Study the drawing (mm; zero at the part's minimum x, y, z) and answer. Coordinates: 2 decimals unless noted, no trailing zeros. Loops run counter-clockwise (first coordinate to the right, second up) from the corner with the lowest first, then second, coordinate; pieces in that order, holes last. Notation, with made-up numbers: (26.25, -23) -> (81.25, -23) arc R36 ccw to (81.25, 16) -> close; hole circle Ø1 at (29, -6). An arc over 180 degrees is marked (long way). Answer as a JSON object with one key per item and string values. Group by question number.
Q1. Straight lines are drawn through the part: line 1 along X through (y, z) = (11.5, 4.85); line 2 along X through (y, z) = (7.75, 3); line 3 along Y through (x, z) = (17.5, 4) (1 decimal). For each, find the intervals that lie inside material, in ascending order. Write a range as [from, to].
Q2. Each of these flat-tipped pins is pushed along its axis until it touches: P1, Ø1, axis at y = 14, z = 6, coming from the -X side (1 decimal); P2, Ø3, axis at x = 17, y = 5.5, coming from the -Z side; P3, Ø0.7, axis at y = 22, z = 4, coming from the +X side (1 decimal); P4, Ø4, axis at y = 8.5, z = 2.5, coming from the +X side. Where does it stop, or does it pass through?
Q3. The part is cut by section C-C on z = 2.5. Write down the section's boundary in (x, y).
Q4. The part is cut by section A-A on y = 11.5. Write down the section's boundary in (x, z), and give its area (3 significant figures).
Q5. The part is cut by section B-B on x = 11.5. Write down the section's boundary in (y, z).
Q6. Determine the mould class of the marked faces 1 and 2 for opening direction Y: released by +Y, released by -Y, zero draft, split by the parting line, or undercut.
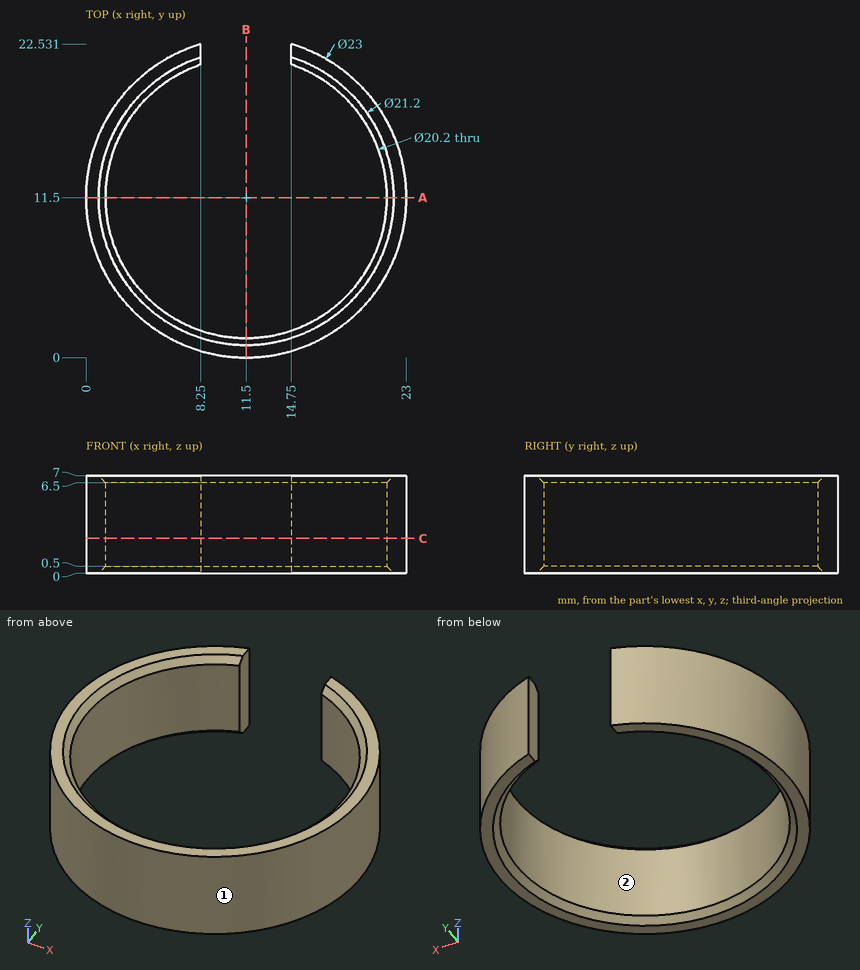
Final values:
{
 "1": {"line 1": "x = [0, 1.4], [21.6, 23]", "line 2": "x = [0.63, 2.12], [20.88, 22.37]", "line 3": "y = [1.7, 3.4], [19.6, 21.3]"},
 "2": {"P1": "stops at x = 0.2", "P2": "passes through", "P3": "stops at x = 16.9", "P4": "stops at x = 22.96"},
 "3": {"outline": "(8.25, 21.06) -> (8.25, 22.53) arc R11.5 ccw (long way) to (14.75, 22.53) -> (14.75, 21.06) arc R10.1 cw (long way) to start"},
 "4": {"outline": "(0, 0) -> (0.9, 0) -> (1.4, 0.5) -> (1.4, 6.5) -> (0.9, 7) -> (0, 7) -> close; (21.6, 0.5) -> (22.1, 0) -> (23, 0) -> (23, 7) -> (22.1, 7) -> (21.6, 6.5) -> close", "area": "19.1 mm2"},
 "5": {"outline": "(0, 0) -> (0.9, 0) -> (1.4, 0.5) -> (1.4, 6.5) -> (0.9, 7) -> (0, 7) -> close"},
 "6": {"face 1": "split by the parting line", "face 2": "undercut"}
}
